from build123d import *

# Parameters (mm, degrees)
SKETCH_1_R      = 35
EXTRUDE_1_DEPTH = 25


with BuildPart() as part:
    # 草图1 → 凸台-拉伸1 (new body)
    with BuildSketch(Plane.XY):
        with BuildLine():
            Line((129, 0), (129, 10))
            Line((129, 10), (100.448181422, 24.59601507))
            ThreePointArc((100.448181422, 24.59601507), (96.470105928, 28.280717759), (95, 33.5))
            Line((95, 33.5), (95, 81.5))
            ThreePointArc((95, 81.5), (87.840181999, 105.854067962), (68.639083275, 122.458327293))
            Line((68.639083275, 122.458327293), (16.907594042, 146))
            Line((16.907594042, 146), (0, 82.9))
            Line((0, 82.9), (0, -22.47))
            Line((0, -22.47), (129, -22.47))
            Line((129, -22.47), (129, 0))
        make_face()
        with Locations((50, 81.5)):
            Circle(SKETCH_1_R, mode=Mode.SUBTRACT)
    extrude(amount=EXTRUDE_1_DEPTH)


solid = part.part
Work out the finished part from the listing and answer in its coordinate system (mm). A direction names the side the tool comes from. Coordinates: 2 decimals unless noted, no trailing zeros. Loops run counter-clockwise (first coordinate to the right, second up) from the corner with the lowest first, then second, coordinate; pieces in that order, holes last. Notation, with made-up numbers: (26.5, -34.75) -> (41.5, -34.75) arc R19 ccw to (41.5, -27.75) -> close; hole circle Ø5 at (72, 51.25). An arc over 180 degrees is marked (long way). Write each question's results on one line, items separated by ' | '. Start each with the question number.
1) For faces 4 (the flat face through (95, 57, 12)), 5 (the flat face through (0, 31, 12)), determine the directions among +Z, -Z, +X, -X, +Y, -Y from which every point of the face is accessible in a straight line to the end or side of a thin tool.
2) Find section C-C on z = 8. Determine the outline of the cut face in (x, y), then the cut area to 3 significant figures.
3) The mould has two halves that part along Y. Classify faces 1 (the flat face through (49, 26, 0)), 2 (the flat face through (64, -22.47, 12)), 3 (the cylindrical face through (24.2, 105.15, 12.32)): pulls with the +Y half, pulls with the -Y half, needs draft (parallel to the pull), parting line crosses it, or undercut.
4) Find section A-A on x = 50. Determine the outline of the cut face in (y, z).
5) Flat-ended cylindrical pins translate along their axes: P1, Ø7.5, axis at y = 52.5, z = 7.5, coming from the +X side; P2, Ø6, axis at x = 94.5, z = 4, coming from the +Y side; P3, Ø3, axis at y = 94, z = 3.5, coming from the -X side. Find the tip coordinate at first contact, or state that the pin passes through.
6) Consider line 1 along Y through (x, z) = (50, 17.75); line 2 along X through (y, z) = (104, 2); line 3 along Y through (x, z) = (38, 16). Determine where each line is inside the solid, lowest interval first.
7) Find section B-B on y = 63.5. Determine the outline of the cut face in (x, z).
8) Find section D-D on y = 36. Determine the outline of the cut face in (x, z), then the cut area to 4 significant figures.
Response values:
1) face 4: +Z, -Z, +X, +Y | face 5: +Z, -Z, -X, +Y, -Y
2) outline: (0, -22.47) -> (129, -22.47) -> (129, 10) -> (100.45, 24.6) arc R10 cw to (95, 33.5) -> (95, 81.5) arc R45 ccw to (68.64, 122.46) -> (16.91, 146) -> (0, 82.9) -> close; hole circle Ø70 at (50, 81.5) | area: 11,500 mm^2
3) face 1: needs draft | face 2: pulls with the -Y half | face 3: undercut
4) outline: (-22.47, 0) -> (46.5, 0) -> (46.5, 25) -> (-22.47, 25) -> close; (116.5, 0) -> (130.94, 0) -> (130.94, 25) -> (116.5, 25) -> close
5) P1: stops at x = 95 | P2: stops at y = 98.9 | P3: stops at x = 2.57
6) line 1: y = -22.47 to 46.5, 116.5 to 130.94 | line 2: x = 5.65 to 23.19, 76.81 to 88.97 | line 3: y = -22.47 to 48.62, 114.38 to 136.4
7) outline: (0, 0) -> (19.98, 0) -> (19.98, 25) -> (0, 25) -> close; (80.02, 0) -> (95, 0) -> (95, 25) -> (80.02, 25) -> close
8) outline: (0, 0) -> (95, 0) -> (95, 25) -> (0, 25) -> close | area: 2,375 mm^2
